Answer from the drawing. Dimensions are ordinates in mm from the lowest x, y and z of the part. A direction names the side the tool comes from. Give positions to 0.01 mm unless a question says otherwise; leave off trailing zeros. Order: outer loops, then holes, each group sorted by start corner. A loop starts at its lowest first (then second) coordinate and runs counter-clockwise, first axis right, second up. Notation, with made-up numbers: (67, 88.5) -> (110, 88.5) arc R25 ccw to (110, 105.5) -> close; hole circle Ø2 at (-27.5, 25). An arc over 180 degrees is marked (long way). Write item = value, one per line. Start each with the question number.
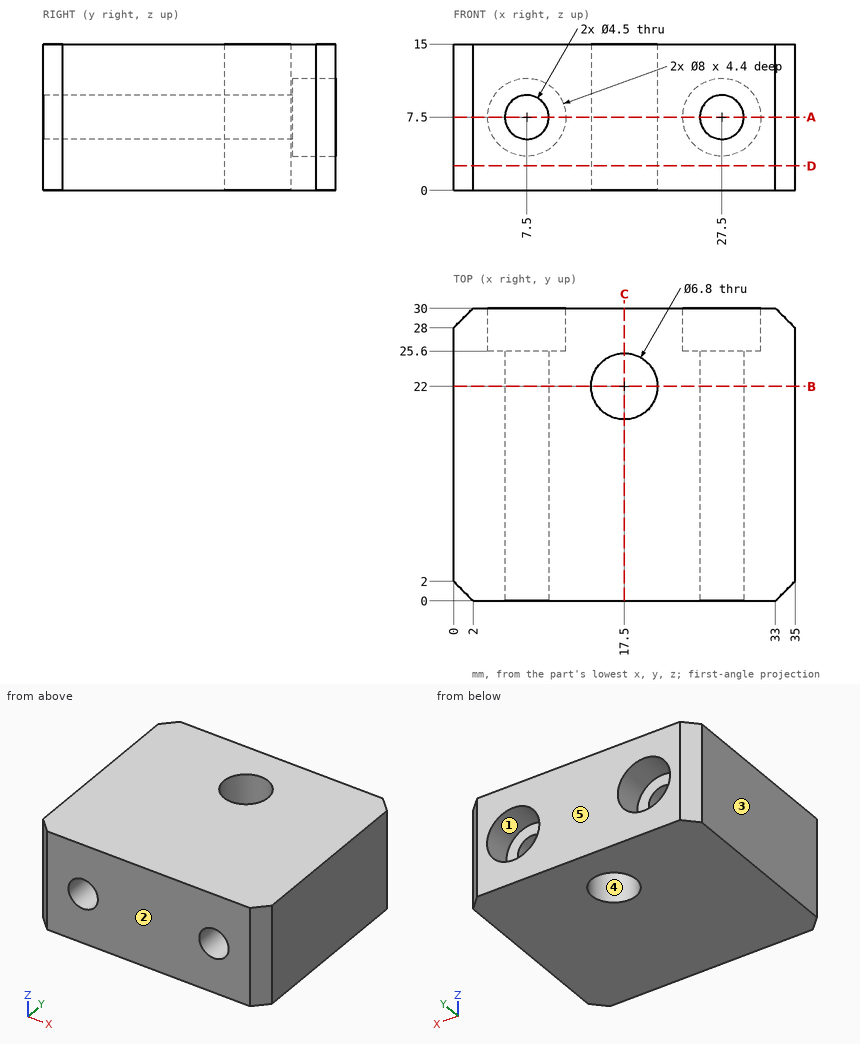
Item 1: A cutting plane is placed at C-C, the plane x = 17.5. Write down the section's boundary in (y, z).
Item 2: The mould has two halves that part along Y. Classify the marked faces 3, 4 and 5: +Y half, -Y half, draft (parallel to the pull), parting line (faces both ways), or undercut.
Item 3: Consider L1, parallel to Z at x = 27.5, y = 9.25; L2, parallel to Z at x = 27.5, y = 27.15; L3, parallel to X at y = 26, z = 8. Determine where each line is inside the solid, lowest interval first. Write a range as from..to.
Item 4: A cutting plane is placed at A-A, the plane z = 7.5. Write down the section's boundary in (x, y).
Item 5: Which of the six approach directions +Z, -Z, +X, -X, +Y, -Y give full straight-line access (tool end or side, diameter ignored) to the marked faces 1 and 2?
Item 6: A cutting plane is placed at D-D, the plane z = 2.5. Write down the section's boundary in (x, y).
Item 7: A cutting plane is placed at B-B, the plane y = 22. Write down the section's boundary in (x, z), plus the area to 3 significant figures.
Check values:
q1.outline = (0, 0) -> (18.6, 0) -> (18.6, 15) -> (0, 15) -> close; (25.4, 0) -> (30, 0) -> (30, 15) -> (25.4, 15) -> close
q2.face_3 = draft
q2.face_4 = undercut
q2.face_5 = +Y half
q3.L1 = 0..5.25, 9.75..15
q3.L2 = 0..3.5, 11.5..15
q3.L3 = 0..3.53, 11.47..23.53, 31.47..35
q4.outline = (0, 2) -> (2, 0) -> (5.25, 0) -> (5.25, 25.6) -> (3.5, 25.6) -> (3.5, 30) -> (2, 30) -> (0, 28) -> close; (9.75, 0) -> (25.25, 0) -> (25.25, 25.6) -> (23.5, 25.6) -> (23.5, 30) -> (11.5, 30) -> (11.5, 25.6) -> (9.75, 25.6) -> close; (29.75, 0) -> (33, 0) -> (35, 2) -> (35, 28) -> (33, 30) -> (31.5, 30) -> (31.5, 25.6) -> (29.75, 25.6) -> close; hole circle Ø6.8 at (17.5, 22)
q5.face_1 = +Y
q5.face_2 = +Z, -Z, +X, -X, -Y
q6.outline = (0, 2) -> (2, 0) -> (33, 0) -> (35, 2) -> (35, 28) -> (33, 30) -> (2, 30) -> (0, 28) -> close; hole circle Ø6.8 at (17.5, 22)
q7.outline = (0, 0) -> (14.1, 0) -> (14.1, 15) -> (0, 15) -> close; (20.9, 0) -> (35, 0) -> (35, 15) -> (20.9, 15) -> close; hole circle Ø4.5 at (7.5, 7.5); hole circle Ø4.5 at (27.5, 7.5)
q7.area = 391 mm^2
